Input: part model. Units: mm. Frame: model coordinates. A direction names the side the tool comes from. Give positions to 0.01 mm unless a question says otherwise; leave off trailing zeros. Loops run counter-clockwise (first coordinate to the right, second up) from the corner with the lowest first, then second, coordinate; pieces in that order, holes last. Notation, with made-up numbers: (60, 5) - (69, 5) arc R29 ccw to (69, 42) - close; hole circle Ø9 at (-35, -25.5). An arc over 180 degrees is marked (long way). Answer as a JSON object with one key per item and string values.
from build123d import *

# Parameters (mm, degrees)
SKETCH1_W           = 1000
SKETCH1_H           = 1000
BOSS_EXTRUDE1_DEPTH = 30
CUT_EXTRUDE1_DEPTH  = 708.742891169
SKETCH3_R           = 40
CUT_EXTRUDE2_DEPTH  = 708.742891169
SKETCH4_W           = 120
SKETCH4_H           = 40
CUT_EXTRUDE3_DEPTH  = 20
M10_TAPPED_HOLE1_D  = 8.5


with BuildPart() as part:
    # Sketch1 → Boss-Extrude1 (new body)
    with BuildSketch(Plane.XY):
        Rectangle(SKETCH1_W, SKETCH1_H)
    extrude(amount=BOSS_EXTRUDE1_DEPTH)

    # Sketch2 → Cut-Extrude1 (cut, through all)
    with BuildSketch(Plane.XY.offset(30)):
        with BuildLine():
            ThreePointArc((0, 370), (-141.592869975, 341.835427029), (-261.629509039, 261.629509039))
            ThreePointArc((-261.629509039, 261.629509039), (-261.629509039, 233.345237792), (-233.345237792, 233.345237792))
            ThreePointArc((-233.345237792, 233.345237792), (-126.28553268, 304.880245729), (0, 330))
            ThreePointArc((0, 330), (20, 350), (0, 370))
        make_face()
        with BuildLine():
            ThreePointArc((370, 0), (341.835427029, 141.592869975), (261.629509039, 261.629509039))
            ThreePointArc((261.629509039, 261.629509039), (233.345237792, 261.629509039), (233.345237792, 233.345237792))
            ThreePointArc((233.345237792, 233.345237792), (304.880245729, 126.28553268), (330, 0))
            ThreePointArc((330, 0), (350, -20), (370, 0))
        make_face()
        with BuildLine():
            ThreePointArc((0, -370), (141.592869975, -341.835427029), (261.629509039, -261.629509039))
            ThreePointArc((261.629509039, -261.629509039), (261.629509039, -233.345237792), (233.345237792, -233.345237792))
            ThreePointArc((233.345237792, -233.345237792), (126.28553268, -304.880245729), (0, -330))
            ThreePointArc((0, -330), (-20, -350), (0, -370))
        make_face()
        with BuildLine():
            ThreePointArc((-370, 0), (-341.835427029, -141.592869975), (-261.629509039, -261.629509039))
            ThreePointArc((-261.629509039, -261.629509039), (-233.345237792, -261.629509039), (-233.345237792, -233.345237792))
            ThreePointArc((-233.345237792, -233.345237792), (-304.880245729, -126.28553268), (-330, 0))
            ThreePointArc((-330, 0), (-350, 20), (-370, 0))
        make_face()
    extrude(amount=-CUT_EXTRUDE1_DEPTH, mode=Mode.SUBTRACT)

    # Sketch3 → Cut-Extrude2 (cut, through all)
    with BuildSketch(Plane.XY.offset(30)):
        Circle(SKETCH3_R)
    extrude(amount=-CUT_EXTRUDE2_DEPTH, mode=Mode.SUBTRACT)

    # Sketch4 → Cut-Extrude3 (cut)
    with BuildSketch(Plane.XY.offset(30)):
        with Locations((-90, 0)):
            Rectangle(SKETCH4_W, SKETCH4_H)
        with Locations((90, 0)):
            Rectangle(SKETCH4_W, SKETCH4_H)
    extrude(amount=-CUT_EXTRUDE3_DEPTH, mode=Mode.SUBTRACT)

    # M10 Tapped Hole1 (through all)
    with Locations(Plane.XY.offset(10)):
        with Locations((-130, 0), (-70, 0), (70, 0), (130, 0)):
            Hole(M10_TAPPED_HOLE1_D / 2)


solid = part.part
Item 1: Contact query for flat-ended pins moving along their axis: P1, Ø5, axis at x = 130, y = 0, coming from the +Z side; P2, Ø20, axis at x = 115.5, y = -2, coming from the +Z side. Output: stop coordinate, or through.
Geometry check:
{"P1": "passes through", "P2": "stops at z = 10"}
Item 2: Material intervals for line 1 (Y direction, x = 15.5, z = 20); line 2 (Y direction, x = -92.5, z = 14.75); line 3 (Y direction, x = -22.5, z = 14), sorted ascending. Write a range as [from, to].
Geometry check:
{"line 1": "y = [-500, -369.68], [-329.64, -36.87], [36.87, 337.36], [362.64, 500]", "line 2": "y = [-500, -20], [20, 316.77], [358.25, 500]", "line 3": "y = [-500, -33.07], [33.07, 329.23], [369.32, 500]"}
Item 3: Cut plane C-C (z = 19). Return loops of the section in (x, y), then the cut area to 3 significant figures.
Geometry check:
{"outline": "(-500, -500) - (500, -500) - (500, 500) - (-500, 500) - close; hole (-370, 0) arc R370 ccw to (-261.63, -261.63) arc R20 ccw to (-233.35, -233.35) arc R330 cw to (-330, 0) arc R20 ccw to start; hole (-261.63, 261.63) arc R20 ccw to (-233.35, 233.35) arc R330 cw to (0, 330) arc R20 ccw to (0, 370) arc R370 ccw to start; hole (-150, -20) - (-34.64, -20) arc R40 ccw to (34.64, -20) - (150, -20) - (150, 20) - (34.64, 20) arc R40 ccw to (-34.64, 20) - (-150, 20) - close; hole (0, -370) arc R370 ccw to (261.63, -261.63) arc R20 ccw to (233.35, -233.35) arc R330 cw to (0, -330) arc R20 ccw to start; hole (233.35, 233.35) arc R330 cw to (330, 0) arc R20 ccw to (370, 0) arc R370 ccw to (261.63, 261.63) arc R20 ccw to start", "area": "937,000 mm2"}
Item 4: Cut plane D-D (x = -247). Return loops of the section in (y, z).
Geometry check:
{"outline": "(-500, 0) - (-267.48, 0) - (-267.48, 30) - (-500, 30) - close; (-218.84, 0) - (227.49, 0) - (227.49, 30) - (-218.84, 30) - close; (275.48, 0) - (500, 0) - (500, 30) - (275.48, 30) - close"}
Item 5: Cut plane A-A (y = 350). Return loops of the section in (x, z).
Geometry check:
{"outline": "(-500, 0) - (-120, 0) - (-120, 30) - (-500, 30) - close; (20, 0) - (500, 0) - (500, 30) - (20, 30) - close"}
Item 6: Mould query, pull axis Y, two halves, no side actions, for faces 3 (the face through (-7, -500, 15)), 4 (the face through (-261.94, 233.66, 15.21)), 5 (the face through (500, -7, 15)). Classes: released by +Y, released by -Y, zero draft, split by the parting line, or undercut.
Geometry check:
{"face 3": "released by -Y", "face 4": "undercut", "face 5": "zero draft"}
Item 7: Access query for faces 1 (the face through (-93, 0, 10)), 2 (the face through (-342.61, -139.71, 15.21)). Directions: +Z, -Z, +X, -X, +Y, -Y. A direction counts if a zero-diameter tool reaches every point of the face in a straight line with its end or side. Return the directions, or none.
Geometry check:
{"face 1": "+Z", "face 2": "+Z, -Z"}
